```python
from build123d import *
from build123d.topology import SkipClean

# Parameters (mm, degrees)
BASE_BRACKET_DEPTH        = 30
HUB_BOSS_SKETCH_R         = 30
HUB_BOSS_SKETCH_R_2       = 20
HUB_BOSS_DEPTH            = 60
LUG_ARM_SKETCH_R          = 10
LUG_ARM_DEPTH             = 15
CONNECTING_WEB_SKETCH_W   = 40
CONNECTING_WEB_SKETCH_H   = 10
CONNECTING_WEB_DEPTH      = 30
HUB_START                 = -60
HUB_BORE_SKETCH_R         = 20
HUB_BORE_DEPTH            = 60
SUPPORT_RIB_REACH         = 120.76
SUPPORT_RIB_SKETCH_WALL_W = 296.52928849
SUPPORT_RIB_SKETCH_WALL_H = 10
SIDE_WALL_HOLES_SKETCH_R  = 8
SIDE_WALL_HOLES_DEPTH     = 15


with BuildPart() as part:
    # Base Bracket Profile Sketch → Base Bracket (new, symmetric)
    with BuildSketch(Plane.XY):
        Polygon((0, 15), (-75, 15), (-75, 60), (-60, 60), (-60, 30), (0, 30), align=None)
    extrude(amount=BASE_BRACKET_DEPTH, both=True)

    # Hub Boss Sketch → Hub Boss (add)
    with BuildSketch(Plane(origin=(0, 0, 0), x_dir=(1, 0, 0), z_dir=(0, 1, 0))):
        with Locations(Location((0, 0, 0), (0, 0, 270))):
            Circle(HUB_BOSS_SKETCH_R)
        with Locations(Location((0, 0, 0), (0, 0, 270))):
            Circle(HUB_BOSS_SKETCH_R_2, mode=Mode.SUBTRACT)
    extrude(amount=HUB_BOSS_DEPTH)

    # Lug Arm Sketch → Lug Arm (add)
    with BuildSketch(Plane(origin=(0, 0, 0), x_dir=(1, 0, 0), z_dir=(0, 1, 0))):
        with BuildLine():
            Line((74.999995036, 23.027288115), (19.14580869, 23.096276964))
            Line((19.14580869, 23.096276964), (19.293898223, 5.267398918))
            ThreePointArc((19.293898223, 5.267398918), (20, 0), (19.293898223, -5.267398918))
            Line((19.293898223, -5.267398918), (19.293898223, -22.972711885))
            Line((19.293898223, -22.972711885), (74.999995036, -22.972711885))
            ThreePointArc((74.999995036, -22.972711885), (97.999995036, 0.027288115), (74.999995036, 23.027288115))
        make_face()
        with Locations(Location((74.999995036, 0.027288115, 0), (0, 0, 270))):
            Circle(LUG_ARM_SKETCH_R, mode=Mode.SUBTRACT)
    extrude(amount=LUG_ARM_DEPTH)

    # Connecting Web Sketch → Connecting Web (add)
    with BuildSketch(Plane(origin=(0, 60, 0), x_dir=(1, 0, 0), z_dir=(0, 1, 0))):
        with Locations((-40, 0)):
            Rectangle(CONNECTING_WEB_SKETCH_W, CONNECTING_WEB_SKETCH_H)
    extrude(amount=-CONNECTING_WEB_DEPTH)

    # Hub Bore Sketch → Hub Bore (cut)
    with SkipClean():  # the faces are left unmerged after this step: merging them gives an invalid solid
        with BuildSketch(Plane(origin=(0, 60, 0), x_dir=(1, 0, 0), z_dir=(0, 1, 0)).offset(HUB_START)):
            with Locations(Location((0, 0, 0), (0, 0, 270))):
                Circle(HUB_BORE_SKETCH_R)
        extrude(amount=HUB_BORE_DEPTH, mode=Mode.SUBTRACT)

    # Support Rib Sketch wall → Support Rib (add, up to next)
    with BuildSketch(Plane(origin=(37.5, 37.5, 0), x_dir=(0.613940613515, -0.789352217376, 0), z_dir=(0.789352217376, 0.613940613515, 0)), mode=Mode.PRIVATE) as support_rib_sk1:
        Rectangle(SUPPORT_RIB_SKETCH_WALL_W, SUPPORT_RIB_SKETCH_WALL_H)
    support_rib_tool1 = extrude(support_rib_sk1.sketch, amount=-SUPPORT_RIB_REACH, mode=Mode.PRIVATE) - part.part
    add(support_rib_tool1.solids().sort_by_distance((37.5, 37.5, 0))[0])

    # Side Wall Holes Sketch → Side Wall Holes (cut)
    with SkipClean():  # the faces are left unmerged after this step: merging them gives an invalid solid
        with BuildSketch(Plane.ZY.offset(75)):
            with Locations((-17.5, 45)):
                Circle(SIDE_WALL_HOLES_SKETCH_R)
            with Locations((17.5, 45)):
                Circle(SIDE_WALL_HOLES_SKETCH_R)
        extrude(amount=-SIDE_WALL_HOLES_DEPTH, mode=Mode.SUBTRACT)


solid = part.part
```
CAD build for the part. Positions are in the model's coordinates, mm. A direction names the side the tool comes from. Coordinates: 2 decimals unless noted, no trailing zeros. Loops run counter-clockwise (first coordinate to the right, second up) from the corner with the lowest first, then second, coordinate; pieces in that order, holes last. Notation, with made-up numbers: (13, 26.25) - (38, 26.25) arc R22 cw to (38, 34.25) - close; hole circle Ø1 at (56, -28). An arc over 180 degrees is marked (long way). Return JSON: item names as keys, results as strings.
1. Band-saw the part on A-A (y = 42). Give the cut face in (x, z).
Result:
{"outline": "(-75, -30) - (-60, -30) - (-60, -24.92) - (-75, -24.92) - close; (-75, -10.08) - (-60, -10.08) - (-60, -5) - (-29.58, -5) arc R30 ccw to (29.58, -5) - (34, -5) - (34, 5) - (29.58, 5) arc R30 ccw to (-29.58, 5) - (-60, 5) - (-60, 10.08) - (-75, 10.08) - close; (-75, 24.92) - (-60, 24.92) - (-60, 30) - (-75, 30) - close; hole circle Ø40 at (0, 0)"}
2. Mould opens along Y. For faces 4 (the cylindrical face through (-67.6, 50.4, 11.6)), 5 (the flat face through (-44, 30, -17)), 6 (the cylindrical face through (-19.524, 29.58, -4.336)) say: released by +Y, released by -Y, zero draft, split by the parting line, or undercut.
Result:
{"face 4": "undercut", "face 5": "released by +Y", "face 6": "zero draft"}
3. Band-saw the part on C-C (x = 78). Give the cut face in (y, z).
Result:
{"outline": "(0, -22.83) - (15, -22.83) - (15, -9.57) - (0, -9.57) - close; (0, 9.51) - (15, 9.51) - (15, 22.78) - (0, 22.78) - close"}
4. Band-saw the part on D-D (y = 11.5). Give the cut face in (x, z).
Result:
{"outline": "(19.15, -23.1) - (75, -23.03) arc R23 ccw to (75, 22.97) - (19.29, 22.97) arc R30 ccw (long way) to start; hole circle Ø40 at (0, 0); hole circle Ø20 at (75, -0.03)"}
5. Probe L1, parallel to Z at x = 0, y = 14; L2, parallel to Y at x = -63, z = -17; L3, parallel to X at y = 11.5, z = 8. List the from-to ranges inside material, lowest first. Write a range as from..to.
Result:
{"L1": "z = -30..-20, 20..30", "L2": "y = 15..37.02, 52.98..60", "L3": "x = -28.91..-18.33, 18.33..69.04, 80.96..96.55"}
6. Drop flat-ended pins along their axis: pin 1 (21 mm diameter, centred on y = 45, z = -17.5, fed in from -X); pin 2 (1.5 mm diameter, centred on x = -51.5, z = -1, fed in from -Y); pin 3 (18 mm diameter, centred on x = 75, z = -0.03, fed in from -Y); pin 4 (7.5 mm diameter, centred on x = 49.5, y = 4.5, fed in from +Z). Give the stop position or say it passes through.
Result:
{"pin 1": "stops at x = -75", "pin 2": "stops at y = 15", "pin 3": "passes through", "pin 4": "stops at z = 22.97"}
7. Band-saw the part on B-B (z = -12). Give the cut face in (x, y).
Result:
{"outline": "(-75, 15) - (-27.5, 15) - (-27.5, 0) - (-16, 0) - (-16, 60) - (-27.5, 60) - (-27.5, 30) - (-60, 30) - (-60, 39.19) - (-75, 39.19) - close; (-75, 50.81) - (-60, 50.81) - (-60, 60) - (-75, 60) - close; (16, 0) - (94.64, 0) - (94.64, 15) - (27.5, 15) - (27.5, 60) - (16, 60) - close"}
8. 3-axis set-ups, long thin cutter, end or side, ignore diameter. For faces 1 (the flat face through (36, 27, -5)), 2 (the flat face through (58, 15, 0)), 3 (the flat face through (-45, 45, -5)): which of +Z, -Z, +X, -X, +Y, -Y reach the whole face in a straight line?
Result:
{"face 1": "-Z, +X, +Y", "face 2": "+X, +Y", "face 3": "-Z, +Y"}
